Part model, mm, in its own coordinate system. Face numbers are marked on the shaded views. A direction names the side the tool comes from. Round coordinates to 2 decimals unless told otherwise and drop trailing zeros. Loops run counter-clockwise (first coordinate to the right, second up) from the corner with the lowest first, then second, coordinate; pieces in that order, holes last. Notation, with made-up numbers: M 13,36.25 L 57,36.25 A36 ccw 57,73.25 Z; hole C 80.5,38 d11. An arc over 180 degrees is marked long. Put each result on its own line as item: value. Start each with the question number.
1) Drop flat-ended pins along their axis: pin 1 Ø5 at (x, z) = (-1.5, -19.5) entering from -Y; pin 2 Ø4 at (x, y) = (6, 5) entering from -Z; pin 3 Ø1 at (x, y) = (-6, -31.5) entering from +Z. Give the stop position or say it passes through.
2) Which spindle directions (+Z, -Z, +X, -X, +Y, -Y) get a long thin tool onto all of the face, cutting with end or side? Do the marked faces 1, 2 and 3. Say none if no direction does.
3) Slice it at A-A on x = -3.75. Give the cut face in (y, z), then the cut area to 3 significant figures.
4) Slice it at B-B on z = -10.5. Give the cut face in (x, y).
5) Slice it at C-C on y = -41.5. Give the cut face in (x, z), then the cut area to 3 significant figures.
6) Probe line 1 along Z through (x, y) = (6.5, 48); line 2 along Y through (x, z) = (-7.75, -11.5); line 3 along Y through (x, z) = (-1.75, 18). List the from-to ranges inside material, lowest first.
```python
from build123d import *

# Parameters (mm, degrees)
SKETCH_1_W      = 25
SKETCH_1_H      = 110
EXTRUDE_1_DEPTH = 3
SKETCH_3_W      = 25
SKETCH_3_H      = 2
EXTRUDE_2_DEPTH = 18
SKETCH_4_W      = 25
SKETCH_4_H      = 3
EXTRUDE_3_DEPTH = 30
CHAMFER_1_SIZE  = 3


with BuildPart() as part:
    # 草图1 → 凸台-拉伸1 (new body)
    with BuildSketch(Plane.XY):
        Rectangle(SKETCH_1_W, SKETCH_1_H)
    extrude(amount=EXTRUDE_1_DEPTH)

    # 草图3 → 凸台-拉伸2 (add)
    with BuildSketch(Plane.XY.offset(3)):
        with Locations((0, -54)):
            Rectangle(SKETCH_3_W, SKETCH_3_H)
    extrude(amount=EXTRUDE_2_DEPTH)

    # 草图4 → 凸台-拉伸3 (add)
    with BuildSketch(Plane(origin=(0, 0, 0), x_dir=(-1, 0, 0), z_dir=(0, 0, -1))):
        with Locations((0, 53.5)):
            Rectangle(SKETCH_4_W, SKETCH_4_H)
    extrude(amount=EXTRUDE_3_DEPTH)

    # 倒角1
    chamfer_1_edges = [part.edges().sort_by_distance(p)[0] for p in [
        (-12.5, -54, 21),
        (12.5, -54, 21),
    ]]
    chamfer(chamfer_1_edges, length=CHAMFER_1_SIZE)


solid = part.part
```
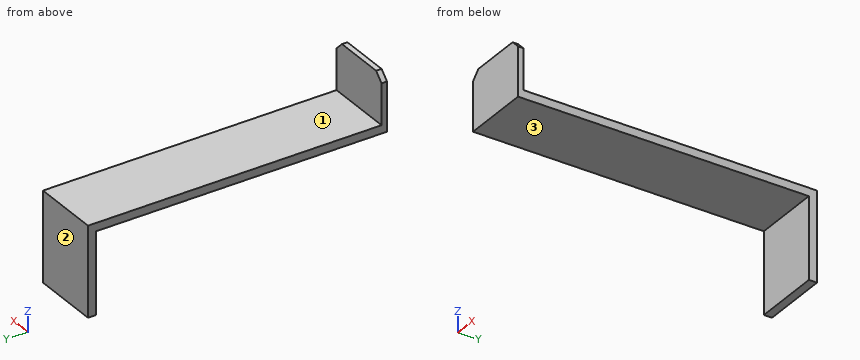
Recorded:
1. pin 1: stops at y = 52
1. pin 2: stops at z = 0
1. pin 3: stops at z = 3
2. face 1: +Z, +X, -X, +Y
2. face 2: +Z, -Z, +X, -X, +Y
2. face 3: -Z, +X, -X, -Y
3. outline: M -55,0 L 52,0 L 52,-30 L 55,-30 L 55,3 L -53,3 L -53,21 L -55,21 Z
3. area: 456 mm2
4. outline: M -12.5,52 L 12.5,52 L 12.5,55 L -12.5,55 Z
5. outline: M -12.5,0 L 12.5,0 L 12.5,3 L -12.5,3 Z
5. area: 75.0 mm2
6. line 1: z = 0 to 3
6. line 2: y = 52 to 55
6. line 3: y = -55 to -53
